from build123d import *

# Parameters (mm, degrees)
SADDLE_BODY_DEPTH     = 40
ARM_TOP_ROUNDS_R20_R  = 20
SIDE_BOSS_DEPTH       = 10
BOSS_POCKET_SKETCH_W  = 20
BOSS_POCKET_SKETCH_H  = 10
BOSS_POCKET_CUT_DEPTH = 25
JOURNAL_BOSS_SKETCH_R = 20
JOURNAL_BOSS_DEPTH    = 40
BASE_SLOT_20X60_DEPTH = 98.979589711
JOURNAL_BORE_SKETCH_R = 13
JOURNAL_BORE_26_DEPTH = 121.0000001


with BuildPart() as part:
    # Saddle Profile Sketch → Saddle Body (new, symmetric)
    with BuildSketch(Plane(origin=(0, 0, 0), x_dir=(0, 0, -1), z_dir=(1, 0, 0))):
        Polygon((-20, 0), (20, 0), (40, 20), (40, 80), (30, 80), (30, 24.142135624), (15.857864376, 10), (-15.857864376, 10), (-30, 24.142135624), (-30, 80), (-40, 80), (-40, 20), align=None)
    extrude(amount=SADDLE_BODY_DEPTH, both=True)

    # Arm Top Rounds R20
    arm_top_rounds_r20_edges = [part.edges().sort_by_distance(p)[0] for p in [
        (-40, 80, 35),
        (-40, 80, -35),
    ]]
    fillet(arm_top_rounds_r20_edges, radius=ARM_TOP_ROUNDS_R20_R)

    # Side Boss Sketch → Side Boss (add)
    with BuildSketch(Plane(origin=(40, 0, 0), x_dir=(0, 0, -1), z_dir=(1, 0, 0))):
        with BuildLine():
            Line((-30, 80), (-22, 80))
            Line((-22, 80), (-22, 38))
            ThreePointArc((-22, 38), (-19.656854249, 32.343145751), (-14, 30))
            Line((-14, 30), (-10, 30))
            Line((-10, 30), (-10, 10))
            Line((-10, 10), (-15.857864376, 10))
            Line((-15.857864376, 10), (-30, 24.142135624))
            Line((-30, 24.142135624), (-30, 80))
        make_face()
        with BuildLine():
            Line((10, 30), (10, 10))
            Line((10, 10), (15.857864376, 10))
            Line((15.857864376, 10), (30, 24.142135624))
            Line((30, 24.142135624), (30, 80))
            Line((30, 80), (22, 80))
            Line((22, 80), (22, 38))
            ThreePointArc((22, 38), (19.656854249, 32.343145751), (14, 30))
            Line((14, 30), (10, 30))
        make_face()
    extrude(amount=-SIDE_BOSS_DEPTH)

    # Boss Pocket Sketch → Boss Pocket Cut (cut)
    with BuildSketch(Plane(origin=(40, 0, 0), x_dir=(0, 0, -1), z_dir=(1, 0, 0))):
        with Locations((0, 5)):
            Rectangle(BOSS_POCKET_SKETCH_W, BOSS_POCKET_SKETCH_H)
    extrude(amount=-BOSS_POCKET_CUT_DEPTH, mode=Mode.SUBTRACT)

    # Journal Boss Sketch → Journal Boss (add)
    with BuildSketch(Plane(origin=(0, 0, 30), x_dir=(-1, 0, 0), z_dir=(0, 0, -1))):
        with Locations(Location((20, 60, 0), (0, 0, 90))):
            Circle(JOURNAL_BOSS_SKETCH_R)
    extrude(amount=JOURNAL_BOSS_DEPTH)

    # Base Slot Sketch → Base Slot 20x60 (cut, through all)
    with BuildSketch(Plane(origin=(0, 0, 0), x_dir=(0, 0, -1), z_dir=(1, 0, 0))):
        with BuildLine():
            Line((0, 70), (14.531264235, 70))
            Line((14.531264235, 70), (14.531264235, 50))
            Line((14.531264235, 50), (0, 50))
            ThreePointArc((0, 50), (-10, 60), (0, 70))
        make_face()
    extrude(amount=-BASE_SLOT_20X60_DEPTH, mode=Mode.SUBTRACT)

    # Journal Bore Sketch → Journal Bore Ø26 (cut, through all)
    with BuildSketch(Plane(origin=(0, 0, -40), x_dir=(-1, 0, 0), z_dir=(0, 0, -1))):
        with Locations((20, 60)):
            Circle(JOURNAL_BORE_SKETCH_R)
    extrude(amount=-JOURNAL_BORE_26_DEPTH, mode=Mode.SUBTRACT)


solid = part.part
Geometry check sheet. Reference: the model listing, model coordinates, mm. A direction names the side the tool comes from. Round coordinates to 2 decimals unless told otherwise and drop trailing zeros. Loops run counter-clockwise (first coordinate to the right, second up) from the corner with the lowest first, then second, coordinate; pieces in that order, holes last. Notation, with made-up numbers: (39.25, 69) - (95.25, 69) arc R18 cw to (95.25, 80) - close; hole circle Ø3 at (42, -1). An arc over 180 degrees is marked (long way). Answer as CSV lines item,"result".
(1) Set-up check for faces 5 (the face through (-7, 70, -5)), 6 (the face through (35, 59, -22)), 7 (the face through (30.5, 11.5, 10)): record each of +Z, -Z, +X, -X, +Y, -Y from which the full face is reachable in a straight line by a thin tool's end or side.
Output values:
face 5,"+X, -X"
face 6,"+X, -X, +Y"
face 7,"+X, +Y, -Y"
(2) Material ranges on line 1 along Y through (x, z) = (-20, 14); line 2 along Z through (x, y) = (28, 68); line 3 along Y through (x, z) = (-20, -34), recorded low to high.
Output values:
line 1,"y = 0 to 10, 40 to 47, 73 to 80"
line 2,"z = -40 to -30, 30 to 40"
line 3,"y = 14 to 47, 73 to 80"
(3) Cross-section at B-B, the plane y = 75. Enter the section's corners in (x, z).
Output values:
outline,"(-33.23, -40) - (40, -40) - (40, -22) - (30, -22) - (30, -30) - (-33.23, -30) - close; (-33.23, -10) - (-6.77, -10) - (-6.77, 30) - (30, 30) - (30, 22) - (40, 22) - (40, 40) - (-33.23, 40) - close"
(4) Cross-section at D-D, the plane x = -27. Enter the section's corners in (y, z) (3 decimals), and give its area (3 significant figures).
Output values:
outline,"(0, -20) - (20, -40) - (49.046, -40) - (49.046, -30) - (24.142, -30) - (10, -15.858) - (10, 15.858) - (24.142, 30) - (41.265, 30) - (41.265, -10) - (49.046, -10) - (49.046, 40) - (20, 40) - (0, 20) - close; (70.954, -40) - (78.735, -40) - (78.735, -30) - (70.954, -30) - close; (70.954, -10) - (78.735, -10) - (78.735, 40) - (70.954, 40) - close"
area,"2,160 mm²"
(5) Depth check by flat-ended pin: pin 1 Ø8 at (y, z) = (2.5, 2.5) entering from +X; pin 2 Ø5 at (x, z) = (-29.5, -30) entering from +Y (3 decimals); pin 3 Ø22 at (y, z) = (52.5, -15) entering from -X. Enter the tip coordinate at first touch or a pass-through.
Output values:
pin 1,"stops at x = 15"
pin 2,"stops at y = 78.735"
pin 3,"stops at x = -37.32"
(6) Cross-section at A-A, the plane x = 33.5. Enter the section's corners in (y, z).
Output values:
outline,"(0, -20) - (20, -40) - (80, -40) - (80, -22) - (38, -22) arc R8 cw to (30, -14) - (30, -10) - (0, -10) - close; (0, 10) - (30, 10) - (30, 14) arc R8 cw to (38, 22) - (80, 22) - (80, 40) - (20, 40) - (0, 20) - close"
(7) Cross-section at C-C, the plane x = -4. Enter the section's corners in (y, z), and give its area (3 significant figures).
Output values:
outline,"(0, -20) - (20, -40) - (80, -40) - (80, -30) - (24.14, -30) - (10, -15.86) - (10, 15.86) - (24.14, 30) - (48, 30) - (48, -10) - (50, -10) - (50, 0) arc R10 cw to (70, 0) - (70, -10) - (72, -10) - (72, 30) - (80, 30) - (80, 40) - (20, 40) - (0, 20) - close"
area,"2,600 mm²"
(8) Release check for a two-part mould opening along Z. For faces 1 (the face through (1, 50, 40)), 2 (the face through (35.07, 32.406, 19.719)), 3 (the face through (40, 41, 28)), 4 (the face through (35, 30, -12)) record: released by +Z, released by -Z, zero draft, split by the parting line, or undercut.
Output values:
face 1,"released by +Z"
face 2,"undercut"
face 3,"zero draft"
face 4,"undercut"
